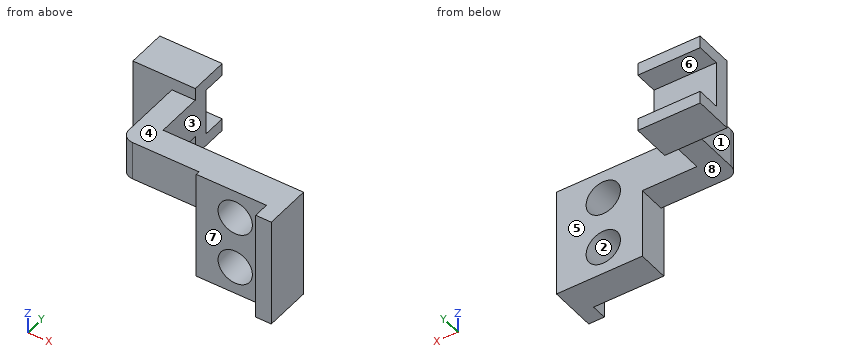
from build123d import *

# Parameters (mm, degrees)
BASE_BRACKET_DEPTH     = 70
UPRIGHT_POST_DEPTH     = 25
SLOTTED_HEAD_DEPTH     = 40
BASE_HOLES_SKETCH_R    = 11
BASE_HOLES_2X_22_DEPTH = 30


with BuildPart() as part:
    # Base Bracket Profile Sketch → Base Bracket (new body)
    with BuildSketch(Plane.XY):
        Polygon((0, 0), (45, 0), (45, -10), (55, -10), (55, 20), (0, 20), align=None)
    extrude(amount=BASE_BRACKET_DEPTH)

    # Upright Post Sketch → Upright Post (add)
    with BuildSketch(Plane.XY.offset(70)):
        with BuildLine():
            Line((-50, 50), (-50, 10))
            ThreePointArc((-50, 10), (-47.803300859, 4.696699141), (-42.5, 2.5))
            Line((-42.5, 2.5), (0, 2.5))
            Line((0, 2.5), (0, 20))
            Line((0, 20), (-35, 20))
            Line((-35, 20), (-35, 50))
            Line((-35, 50), (-50, 50))
        make_face()
    extrude(amount=-UPRIGHT_POST_DEPTH)

    # Slotted Head Profile Sketch → Slotted Head (add)
    with BuildSketch(Plane(origin=(-35, 0, 0), x_dir=(0, 0, -1), z_dir=(1, 0, 0))):
        Polygon((-70, 50), (-78, 50), (-78, 75), (-70, 75), (-70, 60), (-40, 60), (-40, 75), (-32, 75), (-32, 50), align=None)
    extrude(amount=-SLOTTED_HEAD_DEPTH)

    # Base Holes Sketch → Base Holes 2xØ22 (cut)
    with BuildSketch(Plane(origin=(0, 20, 0), x_dir=(1, 0, 0), z_dir=(0, 1, 0))):
        with Locations(Location((25, -18, 0), (0, 0, 270))):
            Circle(BASE_HOLES_SKETCH_R)
        with Locations(Location((25, -52, 0), (0, 0, 270))):
            Circle(BASE_HOLES_SKETCH_R)
    extrude(amount=-BASE_HOLES_2X_22_DEPTH, mode=Mode.SUBTRACT)


solid = part.part
Source: CAD feature listing. Evaluate the final solid. Frame: model axes, mm. Face numbers are marked on the shaded views. A direction names the side the tool comes from. Coordinates: 2 decimals unless noted, no trailing zeros. Order: outer loops, then holes, each group sorted by start corner. A loop starts at its lowest first (then second) coordinate and runs counter-clockwise, first axis right, second up. Notation, with made-up numbers: M -14.5,-7.5 L -0.5,-7.5 A22 cw -0.5,14.5 Z; hole C 9,-27.75 d5. An arc over 180 degrees is marked long. Write each question's results on one line, items separated by ' | '. Start each with the question number.
Item 1: First-contact query: pin 1 Ø20 at (x, z) = (-19, 58) entering from -Y; pin 2 Ø8 at (y, z) = (-2.5, 24.5) entering from -X; pin 3 Ø14 at (x, y) = (-30, 28.5) entering from -Z. Flat tips, straight axial feed; report the tip coordinate or a pass-through.
Item 2: Cut plane D-D (z = 18). Return loops of the section in (x, y).
Item 3: Line query: probe 1 along Z at (x, y) = (-55.5, 71); probe 2 along X at (y, z) = (6, 17.5); probe 3 along Y at (x, z) = (30, 38). Output: solid intervals per line, ascending.
Item 4: Set-up query: the marked faces 5, 6, 7 and 8. Return all of +Z, -Z, +X, -X, +Y, -Y with unobstructed straight access to the full face (end or side cutting, diameter ignored); none if empty.
Item 5: Draft query along X for the marked faces 1, 2, 3 and 4. Return one class per face: pulls with the +X half, pulls with the -X half, needs draft (parallel to the pull), parting line crosses it, or undercut.
Item 6: Cut plane B-B (x = 25). Return loops of the section in (y, z), and give its area (3 significant figures).
Item 7: Cut plane A-A (z = 52). Return loops of the section in (x, y).
Item 8: Cut plane C-C (y = 5.5). Return loops of the section in (x, z).
Checked values:
1) pin 1: stops at y = 2.5 | pin 2: stops at x = 0 | pin 3: stops at z = 45
2) outline: M 0,0 L 14,0 L 14,20 L 0,20 Z; M 36,0 L 45,0 L 45,-10 L 55,-10 L 55,20 L 36,20 Z
3) probe 1: z = 32 to 40, 70 to 78 | probe 2: x = 0 to 14.01, 35.99 to 55 | probe 3: y = 0 to 20
4) face 5: +Z, -Z, +X, +Y | face 6: +X, -X, +Y | face 7: +Z, -Z, -X, -Y | face 8: -Z, -X, -Y
5) face 1: pulls with the -X half | face 2: undercut | face 3: pulls with the +X half | face 4: needs draft
6) outline: M 0,0 L 20,0 L 20,7 L 0,7 Z; M 0,29 L 20,29 L 20,41 L 0,41 Z; M 0,63 L 20,63 L 20,70 L 0,70 Z | area: 520 mm2
7) outline: M -75,50 L -50,50 L -50,10 A7.5 ccw -42.5,2.5 L 0,2.5 L 0,0 L 14,0 L 14,20 L -35,20 L -35,60 L -75,60 Z; M 36,0 L 45,0 L 45,-10 L 55,-10 L 55,20 L 36,20 Z
8) outline: M -48.5,45 L 0,45 L 0,0 L 55,0 L 55,70 L -48.5,70 Z; hole C 25,18 d22; hole C 25,52 d22
